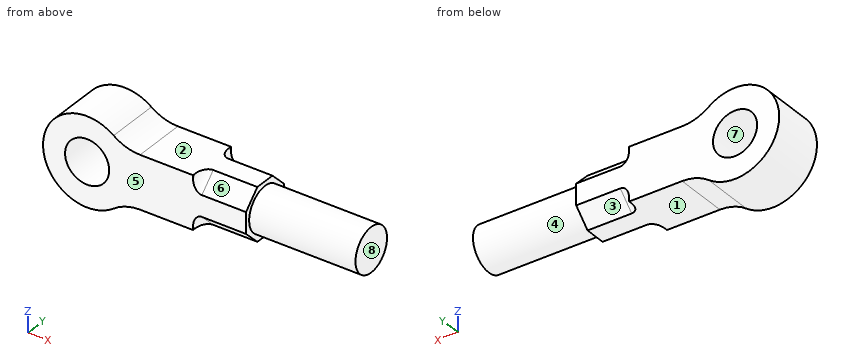
from build123d import *

# Parameters (mm, degrees)
EYE_PROFILE_SKETCH_R   = 25
EYE_BLOCK_60MM_DEPTH   = 60
NECK_FLATS_CUT_DEPTH   = 60
SKETCH2_4_R            = 25
ROD_BOSS_120_5MM_DEPTH = 120.5
NECK_FILLET_R10_R      = 10


with BuildPart() as part:
    # Eye Profile Sketch → Eye Block 60mm (new body)
    with BuildSketch(Plane(origin=(0, 0, 0), x_dir=(1, 0, 0), z_dir=(0, 1, 0))):
        with BuildLine():
            Line((60, 30), (180, 30))
            Line((180, 30), (180, -30))
            Line((180, -30), (60, -30))
            ThreePointArc((60, -30), (44.188611699, -32.565835097), (30, -40))
            ThreePointArc((30, -40), (-50, 0), (30, 40))
            ThreePointArc((30, 40), (44.188611699, 32.565835097), (60, 30))
        make_face()
        with Locations(Location((0, 0, 0), (0, 0, 270))):
            Circle(EYE_PROFILE_SKETCH_R, mode=Mode.SUBTRACT)
    extrude(amount=EYE_BLOCK_60MM_DEPTH)

    # Neck and Rod Sketch → Neck Flats Cut (cut)
    with BuildSketch(Plane(origin=(180, 0, 0), x_dir=(0, 0, -1), z_dir=(1, 0, 0))):
        Polygon((-11.94, 60), (-30, 60), (-30, 41.94), align=None)
        Polygon((30, 60), (11.94, 60), (30, 41.94), align=None)
        Polygon((-11.94, 0), (-30, 18.06), (-30, 0), align=None)
        Polygon((30, 0), (30, 18.06), (11.94, 0), align=None)
    extrude(amount=-NECK_FLATS_CUT_DEPTH, mode=Mode.SUBTRACT)

    # Sketch2_4 → Rod Boss 120.5mm (add)
    with BuildSketch(Plane(origin=(180, 0, 0), x_dir=(0, 0, -1), z_dir=(1, 0, 0))):
        with Locations((0, 30)):
            Circle(SKETCH2_4_R)
    extrude(amount=ROD_BOSS_120_5MM_DEPTH)

    # Neck Fillet R10
    neck_fillet_r10_edges = [part.edges().sort_by_distance(p)[0] for p in [
        (120, 50.97, -20.97),
        (120, 9.03, 20.97),
        (120, 9.03, -20.97),
        (120, 50.97, 20.97),
    ]]
    fillet(neck_fillet_r10_edges, radius=NECK_FILLET_R10_R)


solid = part.part
Here's how the part is built. I have some questions about the finished solid (model axes, mm). Face numbers are marked on the shaded views. A direction names the side the tool comes from. Coordinates: 2 decimals unless noted, no trailing zeros. Write each loop counter-clockwise with the first axis right and the second up, starting at its lowest first coordinate (ties: lowest second). Pieces come first, ordered by that corner, then holes.
1) If we section it at B-B (z = 0): List the corners of the cut face in (x, y) for me.
Filled in:
outline: (-50, 0) - (-25, 0) - (-25, 60) - (-50, 60) - close; (25, 0) - (180, 0) - (180, 5) - (300.5, 5) - (300.5, 55) - (180, 55) - (180, 60) - (25, 60) - close
2) Thinking about a two-plate mould opening in X: for the marked faces 6, 7 and 8, which applies, +X half, -X half, draft (parallel to the pull), parting line (faces both ways), or undercut?
Filled in:
face 6: draft
face 7: undercut
face 8: +X half
3) I'm going to push flat-ended pins straight in: pin 1 (1 mm diameter, centred on y = 32.5, z = 26.5, fed in from +X); pin 2 (12 mm diameter, centred on x = 157.5, y = 32.5, fed in from -Z); pin 3 (8 mm diameter, centred on x = 51.5, y = 26.5, fed in from +Z). Where does each tip first touch, or does it pass through?
Filled in:
pin 1: stops at x = 180
pin 2: stops at z = -30
pin 3: stops at z = 31.59
4) If we section it at C-C (y = 30): List the corners of the cut face in (x, z) for me, plus the area to 3 significant figures.
Filled in:
outline: (30, -40) arc R50 cw to (60, -30) - (180, -30) - (180, -25) - (300.5, -25) - (300.5, 25) - (180, 25) - (180, 30) - (60, 30) arc R50 cw to (30, 40) arc R50 ccw (long way) to start; hole circle Ø50 at (0, 0)
area: 20,000 mm2
5) If we section it at D-D (x = 141): List the corners of the cut face in (y, z) for me, plus the area to 3 significant figures.
Filled in:
outline: (0, -11.94) - (18.06, -30) - (41.94, -30) - (60, -11.94) - (60, 11.94) - (41.94, 30) - (18.06, 30) - (0, 11.94) - close
area: 2,950 mm2
6) Which directions (+Z, -Z, +X, -X, +Y, -Y) give clear straight access to the entire face, cutting with the end or side of a thin tool? Please do the marked faces 1, 2, 3, 4 and 5.
Filled in:
face 1: -Z, +X, +Y, -Y
face 2: +Z, +X, +Y, -Y
face 3: -Z, +X, +Y
face 4: +X
face 5: +Z, -Z, +X, -X, -Y
7) If I drill on line 1 (X direction, y = 6.5, z = 1.5); line 2 (Z direction, x = 91, y = 49.5); line 3 (X direction, y = 28, z = 8.5), over which ranges is the centre line in solid material (lowest first)?
Filled in:
line 1: x = -49.98 to -24.95, 24.95 to 300.5
line 2: z = -30 to 30
line 3: x = -49.27 to -23.51, 23.51 to 300.5
8) If we section it at A-A (x = 0): List the corners of the cut face in (y, z) for me, plus the area to 3 significant figures.
Filled in:
outline: (0, -50) - (60, -50) - (60, -25) - (0, -25) - close; (0, 25) - (60, 25) - (60, 50) - (0, 50) - close
area: 3,000 mm2
